from build123d import *

# Parameters (mm, degrees)
SKETCH_1_W             = 70
SKETCH_1_H             = 80
EXTRUDE_1_DEPTH        = 12
CHAMFER_1_SIZE         = 1
CUT_EXTRUDE_1_DEPTH    = 2.5
PATTERN_LINEAR_1_COUNT = 8
PATTERN_LINEAR_1_PITCH = 10
HOLE_WIZARD_7_0_7_1_D  = 7


with BuildPart() as part:
    # 草图1 → 凸台-拉伸1 (new body)
    with BuildSketch(Plane.XY):
        with Locations((35, -40)):
            Rectangle(SKETCH_1_W, SKETCH_1_H)
    extrude(amount=EXTRUDE_1_DEPTH)

    # 倒角1
    chamfer_1_edges = [part.edges().sort_by_distance(p)[0] for p in [
        (0, 0, 6),
        (70, 0, 6),
        (70, -80, 6),
        (0, -80, 6),
    ]]
    chamfer(chamfer_1_edges, length=CHAMFER_1_SIZE)

    # 草图2 → 切除-拉伸1 (cut)
    with BuildSketch(Plane.XY.offset(12)):
        with BuildLine():
            Line((17.5, -2.5), (52.5, -2.5))
            ThreePointArc((52.5, -2.5), (55, -5), (52.5, -7.5))
            Line((52.5, -7.5), (17.5, -7.5))
            ThreePointArc((17.5, -7.5), (15, -5), (17.5, -2.5))
        make_face()
    cut_extrude_1 = extrude(amount=-CUT_EXTRUDE_1_DEPTH, mode=Mode.SUBTRACT)

    # 阵列(线性)1: 切除-拉伸1 ×8
    with Locations(*[(0, -i * PATTERN_LINEAR_1_PITCH, 0) for i in range(1, PATTERN_LINEAR_1_COUNT)]):
        add(cut_extrude_1, mode=Mode.SUBTRACT)

    # Ø7.0 (7) 直径孔1 (through all)
    with Locations(Plane(origin=(0, 0, 0), x_dir=(-1, 0, 0), z_dir=(0, 0, -1))):
        with Locations((-7, -73), (-7, -7), (-63, -73), (-63, -7)):
            Hole(HOLE_WIZARD_7_0_7_1_D / 2)


solid = part.part
Design review of the part built by this model. Coordinates are the model's own, in mm. A direction names the side the tool comes from. Give positions to 0.01 mm unless a question says otherwise; leave off trailing zeros. Loops run counter-clockwise (first coordinate to the right, second up) from the corner with the lowest first, then second, coordinate; pieces in that order, holes last. Notation, with made-up numbers: M 32.5,67.5 L 66.5,67.5 A27 ccw 66.5,106.5 Z; hole C 10.5,-38 d4. An arc over 180 degrees is marked long. One line per question, with ' | ' between items. Start each with the question number.
1. To check wall thickness, follow L1, parallel to Y at x = 63, z = 8; L2, parallel to Y at x = 65, z = 3.25; L3, parallel to X at y = -25, z = 10.5. State the ranges of each line that lie inside material, in increasing order.
2. Add section D-D (y = -75). Write out the cut boundary in (x, z).
3. For faces 1 (the face through (35, -39, 0)), 2 (the face through (35, -67.5, 11)), list the 3-axis set-ups (+Z, -Z, +X, -X, +Y, -Y) from which the entire face can be reached by the end or side of a thin tool; tool diameter is ignored.
4. The part is to be moulded in two halves that separate along Y. For faces 3 (the face through (35, -39, 12)), 4 (the face through (35, 0, 6)), 5 (the face through (6.241, -76.417, 6.084)), 6 (the face through (15, -65, 11)), say which applies: released by +Y, released by -Y, zero draft, split by the parting line, or undercut.
5. Add section A-A (x = 63). Write out the cut boundary in (y, z), plus the area to 3 significant figures.
6. Insertion check: P1, Ø2.5, axis at x = 33, y = -5.5, coming from the +Z side; P2, Ø6.5, axis at x = 63, y = -7, coming from the +Z side. Each pin has a flat end and moves straight along its axis. Give the tip position at first contact, or say it passes through.
7. Add section C-C (y = -25). Write out the cut boundary in (x, z), plus the area to 3 significant figures.
8. Add section B-B (z = 2.75). Write out the cut boundary in (x, y), plus the area to 3 significant figures.
Worked out:
1) L1: y = -80 to -76.5, -69.5 to -10.5, -3.5 to 0 | L2: y = -80 to -75.87, -70.13 to -9.87, -4.13 to 0 | L3: x = 0 to 15, 55 to 70
2) outline: M 0,0 L 4.13,0 L 4.13,12 L 0,12 Z; M 9.87,0 L 60.13,0 L 60.13,12 L 55,12 L 55,9.5 L 15,9.5 L 15,12 L 9.87,12 Z; M 65.87,0 L 70,0 L 70,12 L 65.87,12 Z
3) face 1: -Z, +X, -X, +Y, -Y | face 2: +Z
4) face 3: zero draft | face 4: released by +Y | face 5: undercut | face 6: undercut
5) outline: M -80,0 L -76.5,0 L -76.5,12 L -80,12 Z; M -69.5,0 L -10.5,0 L -10.5,12 L -69.5,12 Z; M -3.5,0 L 0,0 L 0,12 L -3.5,12 Z | area: 792 mm²
6) P1: stops at z = 9.5 | P2: passes through
7) outline: M 0,0 L 70,0 L 70,12 L 55,12 L 55,9.5 L 15,9.5 L 15,12 L 0,12 Z | area: 740 mm²
8) outline: M 0,-79 L 1,-80 L 69,-80 L 70,-79 L 70,-1 L 69,0 L 1,0 L 0,-1 Z; hole C 7,-73 d7; hole C 7,-7 d7; hole C 63,-73 d7; hole C 63,-7 d7 | area: 5,440 mm²
